from build123d import *

# Parameters (mm, degrees)
SKETCH1_W                                            = 34
SKETCH1_H                                            = 14
BOSS_EXTRUDE1_DEPTH                                  = 10
HOLE_SIZE_PER_SOCKET_HEAD_CAP_SCREW_TYPE_D           = 5.5
HOLE_SIZE_PER_SOCKET_HEAD_CAP_SCREW_TYPE_CBORE_D     = 10
HOLE_SIZE_PER_SOCKET_HEAD_CAP_SCREW_TYPE_CBORE_DEPTH = 5.7
BOSS_EXTRUDE2_DEPTH                                  = 10
CHAMFER2_SIZE                                        = 2
CHAMFER1_SIZE                                        = 0.5


with BuildPart() as part:
    # Sketch1 → Boss-Extrude1 (new body)
    with BuildSketch(Plane.XY):
        Rectangle(SKETCH1_W, SKETCH1_H)
    extrude(amount=BOSS_EXTRUDE1_DEPTH)

    # Hole size per socket head cap screw type1 (through all)
    with Locations(Plane(origin=(-10, 0, 10), x_dir=(1, 0, 0), z_dir=(0, 0, 1))):
        with Locations((0, 0), (20, 0)):
            CounterBoreHole(HOLE_SIZE_PER_SOCKET_HEAD_CAP_SCREW_TYPE_D / 2, HOLE_SIZE_PER_SOCKET_HEAD_CAP_SCREW_TYPE_CBORE_D / 2, HOLE_SIZE_PER_SOCKET_HEAD_CAP_SCREW_TYPE_CBORE_DEPTH)

    # Sketch3 → Boss-Extrude2 (add)
    with BuildSketch(Plane.XY.offset(10)):
        Polygon((-17, -7), (-5, -26), (5, -26), (17, -7), align=None)
    extrude(amount=-BOSS_EXTRUDE2_DEPTH)

    # Chamfer2
    chamfer2_edges = [part.edges().sort_by_distance(p)[0] for p in [
        (-17, 7, 5),
        (17, 7, 5),
    ]]
    chamfer(chamfer2_edges, length=CHAMFER2_SIZE)

    # Chamfer1
    chamfer1_edges = [part.edges().sort_by_distance(p)[0] for p in [
        (17, -1, 10),
        (5, 0, 10),
        (12.75, 0, 0),
        (-15, 0, 10),
        (-7.25, 0, 0),
        (-11, -16.5, 10),
        (0, -26, 10),
        (11, -16.5, 10),
        (11, -16.5, 0),
        (0, -26, 0),
        (-11, -16.5, 0),
        (-17, -1, 0),
        (-17, -1, 10),
        (0, 7, 0),
        (16, 6, 0),
        (-16, 6, 0),
        (0, 7, 10),
        (16, 6, 10),
        (-16, 6, 10),
        (17, -1, 0),
    ]]
    chamfer(chamfer1_edges, length=CHAMFER1_SIZE)


solid = part.part
Work out the finished part from the listing and answer in its coordinate system (mm). A direction names the side the tool comes from. Round coordinates to 2 decimals unless told otherwise and drop trailing zeros. Write each loop counter-clockwise with the first axis right and the second up, starting at its lowest first coordinate (ties: lowest second). Pieces come first, ordered by that corner, then holes. Notation, with made-up numbers: M -6.75,-1.75 L 36.25,-1.75 A17 ccw 36.25,25.25 Z; hole C 21.25,13.5 d1. An arc over 180 degrees is marked long. Use a Markdown table: item, result.
1) Which of the six approach directions +Z, -Z, +X, -X, +Y, -Y give full straight-line access (tool end or side, diameter ignored) to faces 1 (the face through (12.2, -2.2, 4.3)), 2 (the face through (0, -6, 0))?
Taken from the geometry:
| item | result |
|---|---|
| face 1 | +Z |
| face 2 | -Z, +X, -X, +Y, -Y |
2) Determine the mould class of faces 3 (the face through (10.92, -16.63, 5.06)), 4 (the face through (-17, -1, 5)), 5 (the face through (14.77, 1.5, 6.94)), 6 (the face through (0, 7, 5)) for opening direction X: pulls with the +X half, pulls with the -X half, needs draft (parallel to the pull), parting line crosses it, or undercut.
Taken from the geometry:
| item | result |
|---|---|
| face 3 | pulls with the +X half |
| face 4 | pulls with the -X half |
| face 5 | undercut |
| face 6 | needs draft |
3) Consider line 1 (X direction, y = -2.5, z = 7.5); line 2 (X direction, y = -3, z = 7.75); line 3 (Z direction, x = 10, y = -3.5). Determine where each line is inside the solid, lowest interval first. Write a range as [from, to].
Taken from the geometry:
| item | result |
|---|---|
| line 1 | x = [-17, -14.33], [-5.67, 5.67], [14.33, 17] |
| line 2 | x = [-17, -14], [-6, 6], [14, 17] |
| line 3 | z = [0, 4.3] |
4) The part is cut by section C-C on x = 10. Give the vertices of the cut face in (y, z).
Taken from the geometry:
| item | result |
|---|---|
| outline | M -18.08,0.5 L -17.15,0 L -3.25,0 L -2.75,0.5 L -2.75,4.3 L -5,4.3 L -5,9.5 L -5.5,10 L -17.15,10 L -18.08,9.5 Z; M 2.75,0.5 L 3.25,0 L 6.5,0 L 7,0.5 L 7,9.5 L 6.5,10 L 5.5,10 L 5,9.5 L 5,4.3 L 2.75,4.3 Z |
5) The part is cut by section D-D on z = 7.5. Give the vertices of the cut face in (x, y).
Taken from the geometry:
| item | result |
|---|---|
| outline | M -17,-7 L -5,-26 L 5,-26 L 17,-7 L 17,5 L 15,7 L -15,7 L -17,5 Z; hole C -10,0 d10; hole C 10,0 d10 |
6) The part is cut by section B-B on z = 2.75. Give the vertices of the cut face in (x, y).
Taken from the geometry:
| item | result |
|---|---|
| outline | M -17,-7 L -5,-26 L 5,-26 L 17,-7 L 17,5 L 15,7 L -15,7 L -17,5 Z; hole C -10,0 d5.5; hole C 10,0 d5.5 |
7) Flat-ended cylindrical pins translate along their axes: pin 1 (8 mm diameter, centred on x = -10, y = 0, fed in from -Z); pin 2 (2 mm diameter, centred on y = -18, z = 3.5, fed in from +X); pin 3 (1 mm diameter, centred on y = -21.5, z = 8.5, fed in from -X); pin 4 (1.5 mm diameter, centred on x = 10, y = -22.5, fed in from -Z). Find the tip coordinate at first contact, or state that the pin passes through.
Taken from the geometry:
| item | result |
|---|---|
| pin 1 | stops at z = 0 |
| pin 2 | stops at x = 10.68 |
| pin 3 | stops at x = -8.16 |
| pin 4 | passes through |
8) The part is cut by section A-A on y = 0. State how many separate pieces and enclosed holes the cut face has, plus the area to 3 significant figures.
Taken from the geometry:
| item | result |
|---|---|
| separate pieces | 3 |
| enclosed holes | 0 |
| area | 177 mm2 |
